Geometry: final body of the model. Coordinates: model frame, mm. A direction names the side the tool comes from. Round coordinates to 2 decimals unless told otherwise and drop trailing zeros. Order: outer loops, then holes, each group sorted by start corner. A loop starts at its lowest first (then second) coordinate and runs counter-clockwise, first axis right, second up. Notation, with made-up numbers: M 37.5,-29.5 L 71.5,-29.5 A15 cw 71.5,-0.5 Z; hole C 40.25,-38.75 d10. An arc over 180 degrees is marked long. Return JSON: item names as keys, results as strings. Group by question number.
Q1. Cut plane A-A on y = 40. Output: boundary loops of the cut face in (x, z).
Q2. Cut plane B-B on z = 3.5. Output: boundary loops of the cut face in (x, y).
Q3. Cut plane C-C on y = 13. Output: boundary loops of the cut face in (x, z).
Q4. Contact query for flat-ended pins moving along their axis: pin 1 (8.5 mm diameter, centred on x = 11.5, z = -14.5, fed in from -Y); pin 2 (12 mm diameter, centred on x = 46, y = 10, fed in from +Z); pin 3 (5 mm diameter, centred on y = -5.5, z = -16.5, fed in from +X). Output: stop coordinate, or through.
Q5. Cut plane D-D on z = 22. Output: boundary loops of the cut face in (x, y).
Q6. Access query for faces 5 (the face through (37, -10, -4)), 6 (the face through (58, 0, 1)), 7 (the face through (45.7, 19.6, 44.2)), 8 (the face through (52, 42, -2)), 9 (the face through (17, -5, -4)). Directions: +Z, -Z, +X, -X, +Y, -Y. A direction counts if a zero-diameter tool reaches every point of the face in a straight line with its end or side. Return the directions, or none.
Q7. Mould query, pull axis X, two halves, no side actions, for faces 1 (the face through (33, 20, -56.5)), 2 (the face through (66, 25, 1)), 3 (the face through (33, 34, -14)), 4 (the face through (0, 25, 1)). Classes: released by +X, released by -X, zero draft, split by the parting line, or undercut.
Q8. Ray query, probe 1 along X at (y, z) = (19, 3.5); probe 2 along X at (y, z) = (37.5, 50.5); probe 3 along Z at (x, y) = (40, 33). Return the intervals inside material, ascending.
```python
from build123d import *

# Parameters (mm, degrees)
CHANNEL_BLOCK_DEPTH       = 56.5
THROUGH_HOLES_SKETCH_R    = 8
THROUGH_HOLES_2X_16_DEPTH = 98.387114137
SIDE_CUT_DEPTH            = 101.240959692
SIDE_CUT_DEPTH_BACK       = 101.240959692


with BuildPart() as part:
    # Channel Profile Sketch → Channel Block (new, symmetric)
    with BuildSketch(Plane.XY):
        Polygon((0, 0), (0, 50), (14, 50), (14, 34), (52, 34), (52, 50), (66, 50), (66, 0), (49, 0), (49, -10), (17, -10), (17, 0), align=None)
    extrude(amount=CHANNEL_BLOCK_DEPTH, both=True)

    # Through Holes Sketch → Through Holes 2xØ16 (cut, through all)
    with BuildSketch(Plane(origin=(0, 34, 0), x_dir=(1, 0, 0), z_dir=(0, 1, 0))):
        with Locations(Location((33, 34.5, 0), (0, 0, 270))):
            Circle(THROUGH_HOLES_SKETCH_R)
        with Locations(Location((33, -3.5, 0), (0, 0, 270))):
            Circle(THROUGH_HOLES_SKETCH_R)
    extrude(amount=-THROUGH_HOLES_2X_16_DEPTH, mode=Mode.SUBTRACT)

    # Side Cut Sketch → Side Cut (cut, two sides: drawn at the far end of the back side and taken through both)
    with BuildSketch(Plane(origin=(0, 0, 0), x_dir=(1, 0, 0), z_dir=(0, 1, 0)).offset(-SIDE_CUT_DEPTH_BACK)):
        Polygon((-178.698459932, -243.198459932), (8, -56.5), (33, -31.5), (58, -56.5), (244.698459932, -243.198459932), (244.698459932, -771.261448153), (-178.698459932, -771.261448153), align=None)
    extrude(amount=SIDE_CUT_DEPTH + SIDE_CUT_DEPTH_BACK, mode=Mode.SUBTRACT)


solid = part.part
```
Result sheet:
{
 "1": {"outline": "M 0,-56.5 L 14,-56.5 L 14,50.5 L 8,56.5 L 0,56.5 Z; M 52,-56.5 L 66,-56.5 L 66,56.5 L 58,56.5 L 52,50.5 Z"},
 "2": {"outline": "M 0,0 L 17,0 L 17,-10 L 25,-10 L 25,34 L 14,34 L 14,50 L 0,50 Z; M 41,-10 L 49,-10 L 49,0 L 66,0 L 66,50 L 52,50 L 52,34 L 41,34 Z"},
 "3": {"outline": "M 0,-56.5 L 66,-56.5 L 66,56.5 L 58,56.5 L 33,31.5 L 8,56.5 L 0,56.5 Z; hole C 33,-34.5 d16; hole C 33,3.5 d16"},
 "4": {"pin 1": "stops at y = 0", "pin 2": "stops at z = 50.5", "pin 3": "stops at x = 49"},
 "5": {"outline": "M 0,0 L 17,0 L 17,-10 L 49,-10 L 49,0 L 66,0 L 66,50 L 52,50 L 52,34 L 14,34 L 14,50 L 0,50 Z"},
 "6": {"face 5": "+Z, -Z, +X, -X, -Y", "face 6": "+Z, -Z, +X, -Y", "face 7": "+Z, +Y, -Y", "face 8": "+Z, -Z, +Y", "face 9": "+Z, -Z, -X, -Y"},
 "7": {"face 1": "zero draft", "face 2": "released by +X", "face 3": "undercut", "face 4": "released by -X"},
 "8": {"probe 1": "x = 0 to 25, 41 to 66", "probe 2": "x = 0 to 14, 52 to 66", "probe 3": "z = -56.5 to -38.37, -30.63 to -0.37, 7.37 to 38.5"}
}
